Build history of the part. All positions in model axes, mm. Give positions to 0.01 mm unless a question says otherwise; leave off trailing zeros. Order: outer loops, then holes, each group sorted by start corner. A loop starts at its lowest first (then second) coordinate and runs counter-clockwise, first axis right, second up. Notation, with made-up numbers: (-2.75, 17) -> (33.25, 17) arc R11 ccw to (33.25, 24) -> close; hole circle Ø2 at (-32, 72). An arc over 180 degrees is marked (long way). One line per item, written item: value. Start each with the question number.
(1) Saw through at B-B on x = 0. Give the cut face in (y, z), plus the area to 3 significant figures.
(2) Saw through at D-D on x = 7. Give the cut face in (y, z), plus the area to 3 significant figures.
(3) Saw through at C-C on z = 0.95. Give the cut face in (x, y), plus the area to 3 significant figures.
(4) Pin check, flat tips, straight feed: pin 1 (4 mm diameter, centred on x = -7.82, y = -0.82, fed in from -Z); pin 2 (3.5 mm diameter, centred on x = 0, y = 0, fed in from -Z); pin 3 (2 mm diameter, centred on y = -6.5, z = 2.5, fed in from +X); pin 4 (1.5 mm diameter, centred on x = 2, z = 4, fed in from +Y). Stop position of each tip, or through.
(5) Probe line 1 (X direction, y = -0.5, z = 3.25); line 2 (Y direction, x = 0, z = 2.9); line 3 (Z direction, x = -2.5, y = -8.25). List the from-to ranges inside material, lowest first.
(6) Saw through at A-A on y = 7.25. Give the cut face in (x, z), plus the area to 3 significant figures.
(7) Two-plate mould, pull along X, no slides. Class faces 1 (the cylindrical face through (-1.143, 5.536, 3.768)), 2 (the cylindrical face through (-0.59, 4.46, 1.23)), 3 (the flat face through (0, 5, 2.5)): +X half, -X half, draft (parallel to the pull), parting line (faces both ways), or undercut.
```python
from build123d import *

# Parameters (mm, degrees)
SKETCH3_R                = 4.5
SKETCH3_R_2              = 3
BOSS_EXTRUDE1_DEPTH      = 3
BOSS_EXTRUDE2_DEPTH      = 2
BOSS_EXTRUDE2_DEPTH_BACK = 0.5
SKETCH4_R                = 10
SKETCH4_R_2              = 3
SKETCH5_R                = 1.5
CUT_EXTRUDE1_DEPTH       = 16


with BuildPart() as part:
    # Sketch3 → Boss-Extrude1 (new body)
    with BuildSketch(Plane.XY):
        Circle(SKETCH3_R)
        Circle(SKETCH3_R_2, mode=Mode.SUBTRACT)
    extrude(amount=BOSS_EXTRUDE1_DEPTH)

    # Sketch4 → Boss-Extrude2 (add, two sides: drawn at the far end of the back side and taken through both)
    with BuildSketch(Plane.XY.offset(3).offset(-BOSS_EXTRUDE2_DEPTH_BACK)):
        Circle(SKETCH4_R)
        Circle(SKETCH4_R_2, mode=Mode.SUBTRACT)
    extrude(amount=BOSS_EXTRUDE2_DEPTH + BOSS_EXTRUDE2_DEPTH_BACK)

    # Sketch5 → Cut-Extrude1 (cut, through all)
    with BuildSketch(Plane.XY.offset(5)):
        with Locations((7, 0)):
            Circle(SKETCH5_R)
        with Locations((-0.818126129, 7)):
            Circle(SKETCH5_R)
        with Locations((0, -7.818126129)):
            Circle(SKETCH5_R)
        with Locations((-7.818126129, -0.818126129)):
            Circle(SKETCH5_R)
    extrude(amount=-CUT_EXTRUDE1_DEPTH, mode=Mode.SUBTRACT)


solid = part.part
```
Results below:
1. outline: (-10, 2.5) -> (-9.32, 2.5) -> (-9.32, 5) -> (-10, 5) -> close; (-6.32, 2.5) -> (-4.5, 2.5) -> (-4.5, 0) -> (-3, 0) -> (-3, 5) -> (-6.32, 5) -> close; (3, 0) -> (4.5, 0) -> (4.5, 2.5) -> (5.74, 2.5) -> (5.74, 5) -> (3, 5) -> close; (8.26, 2.5) -> (10, 2.5) -> (10, 5) -> (8.26, 5) -> close
1. area: 28.7 mm²
2. outline: (-7.14, 2.5) -> (-1.5, 2.5) -> (-1.5, 5) -> (-7.14, 5) -> close; (1.5, 2.5) -> (7.14, 2.5) -> (7.14, 5) -> (1.5, 5) -> close
2. area: 28.2 mm²
3. outline: circle Ø9 at (0, 0); hole circle Ø6 at (0, 0)
3. area: 35.3 mm²
4. pin 1: stops at z = 2.5
4. pin 2: passes through
4. pin 3: stops at x = 8.35
4. pin 4: stops at y = 9.92
5. line 1: x = -9.99 to -9.28, -6.35 to -2.96, 2.96 to 5.59, 8.41 to 9.99
5. line 2: y = -10 to -9.32, -6.32 to -3, 3 to 5.74, 8.26 to 10
5. line 3: z = 2.5 to 5
6. outline: (-6.89, 2.5) -> (-2.3, 2.5) -> (-2.3, 5) -> (-6.89, 5) -> close; (0.66, 2.5) -> (6.89, 2.5) -> (6.89, 5) -> (0.66, 5) -> close
6. area: 27.0 mm²
7. face 1: undercut
7. face 2: parting line
7. face 3: draft
